Here's how the part is built. I have some questions about the finished solid (model axes, mm). A direction names the side the tool comes from. Coordinates: 2 decimals unless noted, no trailing zeros. Write each loop counter-clockwise with the first axis right and the second up, starting at its lowest first coordinate (ties: lowest second). Pieces come first, ordered by that corner, then holes. Notation, with made-up numbers: (45, 26) -> (101, 26) arc R9 ccw to (101, 36) -> close; hole circle Ø6 at (-28, 29.5). An arc over 180 degrees is marked (long way). Put each result on its own line as item: value.
```python
from build123d import *

# Parameters (mm, degrees)
BASE_PLATE_SKETCH_R     = 11
BASE_PLATE_DEPTH        = 15
REAR_WALL_SKETCH_W      = 18
REAR_WALL_SKETCH_H      = 82
REAR_WALL_DEPTH         = 39
STEP_BLOCKS_SKETCH_W    = 122
STEP_BLOCKS_SKETCH_H    = 12
STEP_BLOCKS_DEPTH       = 15
BEARING_EAR_1_SKETCH_R  = 14
BEARING_EAR_1_DEPTH     = 22
BEARING_START           = -22
BEARING_EAR_2_SKETCH_R  = 14
BEARING_EAR_2_DEPTH     = 22
SADDLE_CUT_DEPTH        = 22
SADDLE_BOSS_DEPTH       = 28
SADDLE_BOSS_FILLET_R1_R = 1
BASE_EDGE_FILLET_R1_R   = 1


with BuildPart() as part:
    # Base Plate Sketch → Base Plate (new body)
    with BuildSketch(Plane(origin=(0, 0, 0), x_dir=(1, 0, 0), z_dir=(0, 1, 0))):
        with BuildLine():
            Line((70, -18), (70, -41))
            Line((70, -41), (-70, -41))
            Line((-70, -41), (-70, 41))
            Line((-70, 41), (70, 41))
            Line((70, 41), (70, 18))
            ThreePointArc((70, 18), (88, 0), (70, -18))
        make_face()
        with Locations(Location((70, 0, 0), (0, 0, 270))):
            Circle(BASE_PLATE_SKETCH_R, mode=Mode.SUBTRACT)
    extrude(amount=BASE_PLATE_DEPTH)

    # Rear Wall Sketch → Rear Wall (add)
    with BuildSketch(Plane(origin=(0, 15, 0), x_dir=(1, 0, 0), z_dir=(0, 1, 0))):
        with Locations((-61, 0)):
            Rectangle(REAR_WALL_SKETCH_W, REAR_WALL_SKETCH_H)
    extrude(amount=REAR_WALL_DEPTH)

    # Step Blocks Sketch → Step Blocks (add)
    with BuildSketch(Plane(origin=(0, 15, 0), x_dir=(1, 0, 0), z_dir=(0, 1, 0))):
        with Locations((9, 35)):
            Rectangle(STEP_BLOCKS_SKETCH_W, STEP_BLOCKS_SKETCH_H)
        with Locations((9, -35)):
            Rectangle(STEP_BLOCKS_SKETCH_W, STEP_BLOCKS_SKETCH_H)
    extrude(amount=STEP_BLOCKS_DEPTH)

    # Bearing Ear 1 Sketch → Bearing Ear 1 (add)
    with BuildSketch(Plane.XY.offset(41)):
        with BuildLine():
            Line((-5, 78.254792273), (-5, 30))
            Line((-5, 30), (-5, 0))
            Line((-5, 0), (45, 0))
            Line((45, 0), (45, 30))
            Line((45, 30), (45, 78.254792273))
            ThreePointArc((45, 78.254792273), (20, 103.254792273), (-5, 78.254792273))
        make_face()
        with Locations((20, 78.254792273)):
            Circle(BEARING_EAR_1_SKETCH_R, mode=Mode.SUBTRACT)
    extrude(amount=-BEARING_EAR_1_DEPTH)

    # Bearing Ear 2 Sketch → Bearing Ear 2 (add)
    with BuildSketch(Plane(origin=(0, 0, -41), x_dir=(-1, 0, 0), z_dir=(0, 0, -1)).offset(BEARING_START)):
        with BuildLine():
            Line((-45, 78.254792273), (-45, 0))
            Line((-45, 0), (5, 0))
            Line((5, 0), (5, 78.254792273))
            ThreePointArc((5, 78.254792273), (-20, 103.254792273), (-45, 78.254792273))
        make_face()
        with Locations(Location((-20, 78.254792273, 0), (0, 0, 180))):
            Circle(BEARING_EAR_2_SKETCH_R, mode=Mode.SUBTRACT)
    extrude(amount=BEARING_EAR_2_DEPTH)

    # Saddle Cut Sketch → Saddle Cut (cut)
    with BuildSketch(Plane.ZY.offset(70)):
        with BuildLine():
            Line((-14, 54), (14, 54))
            ThreePointArc((14, 54), (0, 40), (-14, 54))
        make_face()
    extrude(amount=-SADDLE_CUT_DEPTH, mode=Mode.SUBTRACT)

    # Saddle Boss Sketch → Saddle Boss (add)
    with BuildSketch(Plane.ZY.offset(70)):
        with BuildLine():
            Line((-14, 54), (-22, 54))
            ThreePointArc((-22, 54), (0, 32), (22, 54))
            Line((22, 54), (14, 54))
            ThreePointArc((14, 54), (0, 40), (-14, 54))
        make_face()
    extrude(amount=-SADDLE_BOSS_DEPTH)

    # Saddle Boss Fillet R1
    saddle_boss_fillet_r1_edges = [part.edges().sort_by_distance(p)[0] for p in [
        (-42, 40, 0),
    ]]
    fillet(saddle_boss_fillet_r1_edges, radius=SADDLE_BOSS_FILLET_R1_R)

    # Base Edge Fillet R1
    base_edge_fillet_r1_edges = [part.edges().sort_by_distance(p)[0] for p in [
        (70, 15, -11),
    ]]
    fillet(base_edge_fillet_r1_edges, radius=BASE_EDGE_FILLET_R1_R)


solid = part.part
```
Item 1: For P1, Ø2, axis at x = -22.5, z = -19, coming from the +Y side; P2, Ø20, axis at x = 70, z = 0, coming from the +Y side; P3, Ø17.5, axis at x = 22.5, z = -14, coming from the +Y side; P4, Ø13.5, axis at x = -51, z = 23.5, coming from the +Y side, each with a flat end and sliding along its axis, tell me the tip position at first contact or that it passes through.
Output:
P1: stops at y = 15
P2: passes through
P3: stops at y = 103.25
P4: stops at y = 54
Item 2: Which directions (+Z, -Z, +X, -X, +Y, -Y) give clear straight access to the entire face, cutting with the end or side of a thin tool? Please do faces 5 (the flat face through (-59, 54, -28)), 6 (the flat face through (-52, 30, 1)), 7 (the flat face through (20, 50, 19)), 8 (the flat face through (-29, 22, -29)), 9 (the flat face through (57, 30, -35)).
Output:
face 5: +Z, -Z, -X, +Y
face 6: none
face 7: +X, +Y
face 8: +Y
face 9: +Z, -Z, +X, +Y
Item 3: Please list where these lines run through material, in increasing order: line 1 along Z through (x, y) = (66.5, 25.5); line 2 along X through (y, z) = (5, 0); line 3 along X through (y, z) = (23.5, 28). Write a range as from..to.
Output:
line 1: z = -41..-29, 29..41
line 2: x = -70..59, 81..88
line 3: x = -70..-52, -5..45
Item 4: If we mould it in two halves opening along Z, with no side actions, what happens to faces 1 (the flat face through (-1, 29, 41)), 2 (the flat face through (1, 29, -41)), 3 (the cylindrical face through (26.46, 65.834, 30.154)), 4 (the flat face through (-29, 22, 29))? For each: released by +Z, released by -Z, zero draft, split by the parting line, or undercut.
Output:
face 1: released by +Z
face 2: released by -Z
face 3: zero draft
face 4: undercut
Item 5: Imagine slicing it at D-D on y = 86. Write out the boundary of the cut face in (x, z).
Output:
outline: (-3.77, -41) -> (8.34, -41) -> (8.34, -19) -> (-3.77, -19) -> close; (-3.77, 19) -> (8.34, 19) -> (8.34, 41) -> (-3.77, 41) -> close; (31.66, -41) -> (43.77, -41) -> (43.77, -19) -> (31.66, -19) -> close; (31.66, 19) -> (43.77, 19) -> (43.77, 41) -> (31.66, 41) -> close
Item 6: Imagine slicing it at B-B on y = 61. Write out the boundary of the cut face in (x, z), then the cut area to 3 significant figures.
Output:
outline: (-5, -41) -> (45, -41) -> (45, -19) -> (-5, -19) -> close; (-5, 19) -> (45, 19) -> (45, 41) -> (-5, 41) -> close
area: 2,200 mm²
Item 7: Imagine slicing it at A-A on z = 0. Write out the boundary of the cut face in (x, y), then the cut area to 3 significant figures.
Output:
outline: (-70, 0) -> (59, 0) -> (59, 14) arc R1 ccw to (58, 15) -> (-52, 15) -> (-52, 32) -> (-42, 32) -> (-42, 39) arc R1 ccw to (-43, 40) -> (-70, 40) -> close; (81, 0) -> (88, 0) -> (88, 15) -> (82, 15) arc R1 ccw to (81, 14) -> close
area: 2,570 mm²
Item 8: Imagine slicing it at C-C on x = 20. Write out the boundary of the cut face in (y, z).
Output:
outline: (0, -41) -> (64.25, -41) -> (64.25, -19) -> (15, -19) -> (15, 19) -> (64.25, 19) -> (64.25, 41) -> (0, 41) -> close; (92.25, -41) -> (103.25, -41) -> (103.25, -19) -> (92.25, -19) -> close; (92.25, 19) -> (103.25, 19) -> (103.25, 41) -> (92.25, 41) -> close
